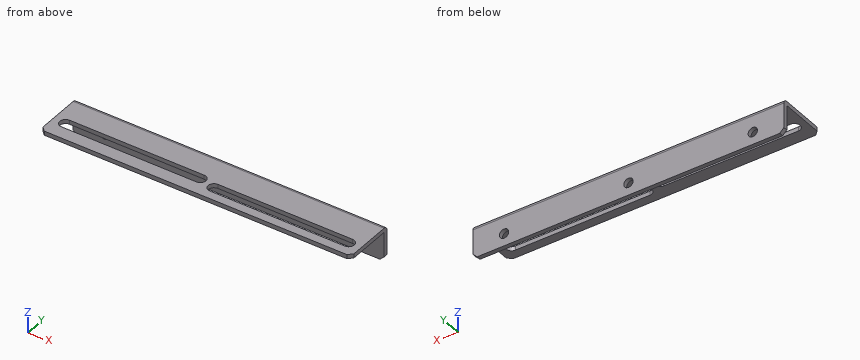
from build123d import *

# Parameters (mm, degrees)
SKETCH_1_W             = 150
SKETCH_1_H             = 25
BOSS_EXTRUDE_1_DEPTH   = 18
SKETCH_2_W             = 16
SKETCH_2_H             = 23
CUT_EXTRUDE_1_DEPTH    = 152.592381075
CUT_EXTRUDE_2_DEPTH    = 78.699742599
CUT_EXTRUDE_3_DEPTH    = 79.136099212
F_4_5_4_5_HOLE_1_D     = 4.5
F_4_5_4_5_HOLE_1_DEPTH = 15
F_4_5_4_5_HOLE_1_TIP   = 1.351936393
F_4_5_4_5_HOLE_3_D     = 4.5
F_4_5_4_5_HOLE_3_DEPTH = 15
F_4_5_4_5_HOLE_3_TIP   = 1.351936393
F_4_5_4_5_HOLE_2_D     = 4.5
F_4_5_4_5_HOLE_2_DEPTH = 15
F_4_5_4_5_HOLE_2_TIP   = 1.351936393
CHAMFER_1_SIZE         = 2
CHAMFER_3_SIZE         = 2
FILLET_1_R             = 2
SKETCH_11_W            = 150
SKETCH_11_H            = 2
CUT_EXTRUDE_4_DEPTH    = 10
CHAMFER_4_SIZE         = 2


with BuildPart() as part:
    # Sketch 1 → Boss-Extrude 1 (new body)
    with BuildSketch(Plane(origin=(0, 0, 0), x_dir=(-1, 0, 0), z_dir=(0, 0, -1))):
        Rectangle(SKETCH_1_W, SKETCH_1_H)
    extrude(amount=-BOSS_EXTRUDE_1_DEPTH)

    # Sketch 2 → Cut-Extrude 1 (cut, through all)
    with BuildSketch(Plane.ZY.offset(75)):
        with Locations((8, -1)):
            Rectangle(SKETCH_2_W, SKETCH_2_H)
    extrude(amount=-CUT_EXTRUDE_1_DEPTH, mode=Mode.SUBTRACT)

    # Sketch 3 → Cut-Extrude 2 (cut, through all)
    with BuildSketch(Plane(origin=(0, 0, 16), x_dir=(-1, 0, 0), z_dir=(0, 0, -1))):
        with BuildLine():
            Line((-4, -2.75), (-69, -2.75))
            ThreePointArc((-69, -2.75), (-71.75, -5.5), (-69, -8.25))
            Line((-69, -8.25), (-4, -8.25))
            ThreePointArc((-4, -8.25), (-1.25, -5.5), (-4, -2.75))
        make_face()
    extrude(amount=-CUT_EXTRUDE_2_DEPTH, mode=Mode.SUBTRACT)

    # Sketch 4 → Cut-Extrude 3 (cut, through all)
    with BuildSketch(Plane.XY.offset(18)):
        with BuildLine():
            Line((-69, -6.25), (-4, -6.25))
            ThreePointArc((-4, -6.25), (-1.25, -3.5), (-4, -0.75))
            Line((-4, -0.75), (-69, -0.75))
            ThreePointArc((-69, -0.75), (-71.75, -3.5), (-69, -6.25))
        make_face()
    extrude(amount=-CUT_EXTRUDE_3_DEPTH, mode=Mode.SUBTRACT)

    # Ø4.5 (4.5) Hole 1
    with Locations(Plane(origin=(0, 12.5, 0), x_dir=(-1, 0, 0), z_dir=(0, 1, 0))):
        with Locations((-60, 8)):
            Hole(F_4_5_4_5_HOLE_1_D / 2, depth=F_4_5_4_5_HOLE_1_DEPTH)
            with Locations((0, 0, -(F_4_5_4_5_HOLE_1_DEPTH + F_4_5_4_5_HOLE_1_TIP / 2))):  # 118° drill point
                Cone(0, F_4_5_4_5_HOLE_1_D / 2, F_4_5_4_5_HOLE_1_TIP, mode=Mode.SUBTRACT)

    # Ø4.5 (4.5) Hole 3
    with Locations(Plane(origin=(0, 12.5, 0), x_dir=(-1, 0, 0), z_dir=(0, 1, 0))):
        with Locations((60, 8)):
            Hole(F_4_5_4_5_HOLE_3_D / 2, depth=F_4_5_4_5_HOLE_3_DEPTH)
            with Locations((0, 0, -(F_4_5_4_5_HOLE_3_DEPTH + F_4_5_4_5_HOLE_3_TIP / 2))):  # 118° drill point
                Cone(0, F_4_5_4_5_HOLE_3_D / 2, F_4_5_4_5_HOLE_3_TIP, mode=Mode.SUBTRACT)

    # Ø4.5 (4.5) Hole 2
    with Locations(Plane(origin=(0, 12.5, 0), x_dir=(-1, 0, 0), z_dir=(0, 1, 0))):
        with Locations((0, 8)):
            Hole(F_4_5_4_5_HOLE_2_D / 2, depth=F_4_5_4_5_HOLE_2_DEPTH)
            with Locations((0, 0, -(F_4_5_4_5_HOLE_2_DEPTH + F_4_5_4_5_HOLE_2_TIP / 2))):  # 118° drill point
                Cone(0, F_4_5_4_5_HOLE_2_D / 2, F_4_5_4_5_HOLE_2_TIP, mode=Mode.SUBTRACT)

    # Chamfer 1
    chamfer_1_edges = [part.edges().sort_by_distance(p)[0] for p in [
        (75, -12.5, 17),
    ]]
    chamfer(chamfer_1_edges, length=CHAMFER_1_SIZE)

    # Chamfer 3
    chamfer_3_edges = [part.edges().sort_by_distance(p)[0] for p in [
        (-75, -12.5, 17),
    ]]
    chamfer(chamfer_3_edges, length=CHAMFER_3_SIZE)

    # Fillet 1
    fillet_1_edges = [part.edges().sort_by_distance(p)[0] for p in [
        (0, 12.5, 18),
    ]]
    fillet(fillet_1_edges, radius=FILLET_1_R)

    # Sketch 11 → Cut-Extrude 4 (cut)
    with BuildSketch(Plane(origin=(0, 12.5, 0), x_dir=(1, 0, 0), z_dir=(0, 1, 0))):
        with Locations((0, -1)):
            Rectangle(SKETCH_11_W, SKETCH_11_H)
    extrude(amount=-CUT_EXTRUDE_4_DEPTH, mode=Mode.SUBTRACT)

    # Chamfer 4
    chamfer_4_edges = [part.edges().sort_by_distance(p)[0] for p in [
        (75, 11.5, 2),
        (-75, 11.5, 2),
    ]]
    chamfer(chamfer_4_edges, length=CHAMFER_4_SIZE)


solid = part.part
Input: part model. Units: mm. Frame: model coordinates. Round coordinates to 2 decimals unless told otherwise and drop trailing zeros. Order: outer loops, then holes, each group sorted by start corner. A loop starts at its lowest first (then second) coordinate and runs counter-clockwise, first axis right, second up.
1. Cut plane D-D, the plane x = 0. Output: boundary loops of the cut face in (y, z), then the cut area to 3 significant figures.
The answers:
outline: (-12.5, 16) - (10.5, 16) - (10.5, 10.25) - (12.5, 10.25) - (12.5, 16) arc R2 ccw to (10.5, 18) - (-12.5, 18) - close; (10.5, 2) - (12.5, 2) - (12.5, 5.75) - (10.5, 5.75) - close
area: 68.1 mm2
2. Cut plane A-A, the plane x = -23. Output: boundary loops of the cut face in (y, z).
The answers:
outline: (-12.5, 16) - (-6.25, 16) - (-6.25, 18) - (-12.5, 18) - close; (-0.75, 16) - (10.5, 16) - (10.5, 2) - (12.5, 2) - (12.5, 16) arc R2 ccw to (10.5, 18) - (-0.75, 18) - close
3. Material intervals for line 1 (Y direction, x = 19.5, z = 15.25); line 2 (Z direction, x = -60, y = 11.4); line 3 (Z direction, x = 51, y = 10), sorted ascending.
The answers:
line 1: y = 10.5 to 12.5
line 2: z = 2 to 5.75, 10.25 to 17.79
line 3: z = 16 to 18
4. Pin query (flat end, axial travel): P1, Ø5, axis at x = 27, y = -9, coming from the -Z side; P2, Ø1.6, axis at x = 43.5, z = 17, coming from the +Y side; P3, Ø8, axis at x = 39.5, z = 9, coming from the -Y side. Return the tip coordinate at first contact, or that it passes through.
The answers:
P1: stops at z = 16
P2: stops at y = 12.49
P3: stops at y = 10.5
5. Cut plane C-C, the plane x = 60. Output: boundary loops of the cut face in (y, z).
The answers:
outline: (-12.5, 16) - (-8.25, 16) - (-8.25, 18) - (-12.5, 18) - close; (-2.75, 16) - (10.5, 16) - (10.5, 10.25) - (12.5, 10.25) - (12.5, 16) arc R2 ccw to (10.5, 18) - (-2.75, 18) - close; (10.5, 2) - (12.5, 2) - (12.5, 5.75) - (10.5, 5.75) - close
6. Cut plane B-B, the plane z = 8. Output: boundary loops of the cut face in (x, y), then the cut area to 3 significant figures.
The answers:
outline: (-75, 10.5) - (-62.25, 10.5) - (-62.25, 12.5) - (-75, 12.5) - close; (-57.75, 10.5) - (-2.25, 10.5) - (-2.25, 12.5) - (-57.75, 12.5) - close; (2.25, 10.5) - (57.75, 10.5) - (57.75, 12.5) - (2.25, 12.5) - close; (62.25, 10.5) - (75, 10.5) - (75, 12.5) - (62.25, 12.5) - close
area: 273 mm2
